The listing builds one solid part. Answer for the finished solid, in the listing's coordinates (mm). Give positions to 0.01 mm unless a question says otherwise; leave off trailing zeros. Write each loop counter-clockwise with the first axis right and the second up, starting at its lowest first coordinate (ties: lowest second). Pieces come first, ordered by that corner, then holes. Notation, with made-up numbers: (-37, 63.5) - (19, 63.5) arc R25 ccw to (19, 101.5) - close; hole circle Ø9 at (41.5, 49.25). An arc over 180 degrees is marked (long way). Write each question's results on one line, items separated by ' | '. Start each with the question number.
Q1. Find the intervals of material crossed by probe 1 along Z at (x, y) = (67.5, -4.5); probe 2 along X at (y, z) = (1, 7.25); probe 3 along Y at (x, z) = (1286, -1.5), in increasing order.
Q2. Flat-ended cylindrical pins translate along their axes: pin 1 Ø0.8 at (y, z) = (7, 1) entering from +X; pin 2 Ø1 at (x, z) = (1210.5, -1) entering from -Y; pin 3 Ø2.5 at (x, z) = (1477.5, 0) entering from +Y. Find the tip coordinate at first contact, or state that the pin passes through.
Q3. Section A-A (x = 159.5) is taken. Determine the outline of the cut face in (y, z).
```python
from build123d import *

# Parameters (mm, degrees)
SKETCH1_R               = 7.5
BOSS_EXTRUDE1_DEPTH     = 1480
CHAMFER1_SIZE           = 1
CUT_EXTRUDE1_DEPTH      = 1481.038006269
CUT_EXTRUDE1_DEPTH_BACK = 1481.038006269
SKETCH8_W               = 43.567276196
SKETCH8_H               = 1.89956865


with BuildPart() as part:
    # Sketch1 → Boss-Extrude1 (new body)
    with BuildSketch(Plane(origin=(0, 0, 0), x_dir=(0, 0, -1), z_dir=(1, 0, 0))):
        Circle(SKETCH1_R)
    extrude(amount=BOSS_EXTRUDE1_DEPTH)

    # Chamfer1
    chamfer1_edges = [part.edges().sort_by_distance(p)[0] for p in [
        (0, 0, 7.5),
        (1480, 0, 7.5),
    ]]
    chamfer(chamfer1_edges, length=CHAMFER1_SIZE)

    # Sketch8 → Cut-Extrude1 (cut, two sides: drawn at the far end of the back side and taken through both)
    with BuildSketch(Plane.XY.offset(-CUT_EXTRUDE1_DEPTH_BACK)):
        with Locations((1492.783638098, 6.949784325)):
            Rectangle(SKETCH8_W, SKETCH8_H)
        with Locations((1492.783638098, -6.949784325)):
            Rectangle(SKETCH8_W, SKETCH8_H)
    extrude(amount=CUT_EXTRUDE1_DEPTH + CUT_EXTRUDE1_DEPTH_BACK, mode=Mode.SUBTRACT)


solid = part.part
```
Answers below:
1) probe 1: z = -6 to 6 | probe 2: x = 0.82 to 1479.18 | probe 3: y = -7.35 to 7.35
2) pin 1: stops at x = 1471 | pin 2: stops at y = -7.48 | pin 3: stops at y = 6
3) outline: circle Ø15 at (0, 0)
